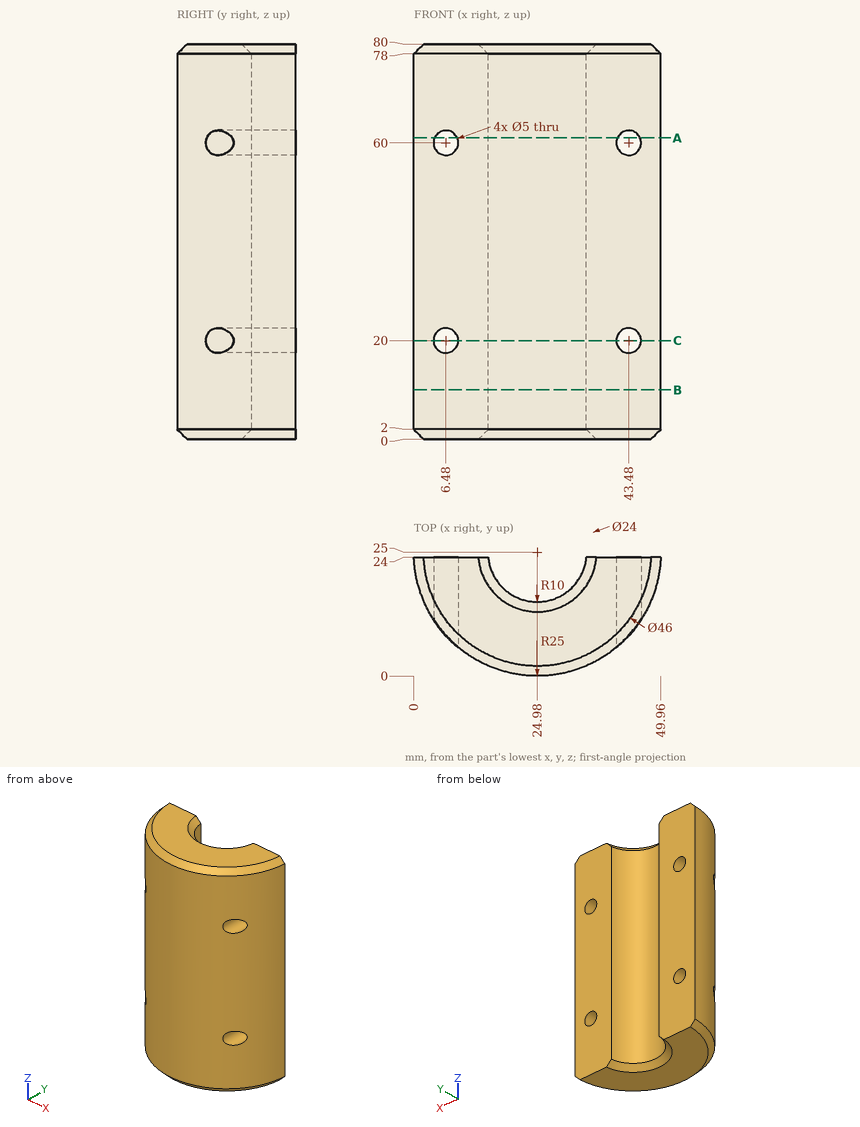
Job drawing, mm, ordinate dimensions from the low corner. One solid piece. Give positions to 0.01 mm unless a question says otherwise; leave off trailing zeros. Order: outer loops, then holes, each group sorted by start corner. A loop starts at its lowest first (then second) coordinate and runs counter-clockwise, first axis right, second up. Notation, with made-up numbers: (-12, 8.5) - (31, 8.5) arc R27 ccw to (31, 42.5) - close; hole circle Ø5 at (-6, 25). An arc over 180 degrees is marked (long way). Answer in a Markdown table with one row per item.
1. Saw through at B-B, the plane z = 10. Give the cut face in (x, y), plus the area to 3 significant figures.
Data:
| item | result |
|---|---|
| outline | (0, 24) arc R25 ccw to (49.96, 24) - (34.93, 24) arc R10 cw to (15.03, 24) - close |
| area | 795 mm² |
2. Flat gauge pins, fed straight in: pin 1 (10 mm diameter, centred on x = 7.5, z = 46.5, fed in from -Y); pin 2 (2 mm diameter, centred on y = 7, z = 39, fed in from -X); pin 3 (4 mm diameter, centred on y = 11.5, z = 24, fed in from +X). Where does each tip first touch, or does it go through?
Data:
| item | result |
|---|---|
| pin 1 | stops at y = 3.34 |
| pin 2 | stops at x = 6.65 |
| pin 3 | stops at x = 47.18 |
3. Saw through at C-C, the plane z = 20. Give the cut face in (x, y).
Data:
| item | result |
|---|---|
| outline | (0, 24) arc R25 ccw to (3.98, 11.44) - (3.98, 24) - close; (8.98, 5.79) arc R25 ccw to (40.98, 5.79) - (40.98, 24) - (34.93, 24) arc R10 cw to (15.03, 24) - (8.98, 24) - close; (45.98, 11.44) arc R25 ccw to (49.96, 24) - (45.98, 24) - close |
4. Saw through at A-A, the plane z = 61. Give the cut face in (x, y).
Data:
| item | result |
|---|---|
| outline | (0, 24) arc R25 ccw to (4.19, 11.12) - (4.19, 24) - close; (8.77, 5.97) arc R25 ccw to (41.19, 5.97) - (41.19, 24) - (34.93, 24) arc R10 cw to (15.03, 24) - (8.77, 24) - close; (45.77, 11.12) arc R25 ccw to (49.96, 24) - (45.77, 24) - close |
5. Probe probe 1 along X at (y, z) = (19.25, 60); probe 2 along X at (y, z) = (17, 20.5); probe 3 along X at (y, z) = (14, 20). List the from-to ranges inside material, lowest first. Write a range as [from, to].
Data:
| item | result |
|---|---|
| probe 1 | x = [0.65, 3.98], [8.98, 16.8], [33.16, 40.98], [45.98, 49.31] |
| probe 2 | x = [1.29, 4.03], [8.93, 18.98], [30.98, 41.03], [45.93, 48.67] |
| probe 3 | x = [2.53, 3.98], [8.98, 40.98], [45.98, 47.43] |
